Check sheet for the modelled part. Datum: model origin and axes. Units: mm. A direction names the side the tool comes from. Give positions to 0.01 mm unless a question says otherwise; leave off trailing zeros. Loops run counter-clockwise (first coordinate to the right, second up) from the corner with the lowest first, then second, coordinate; pieces in that order, holes last. Notation, with made-up numbers: M 56.5,17.5 L 73.5,17.5 A25 cw 73.5,38.5 Z; hole C 45,62 d11. An arc over 180 degrees is marked long. Write each question's results on one line, items separated by ' | '. Start each with the question number.
1. Sectioned sample at A-A on z = 0. Record the cut outline in (x, y).
2. Sectioned sample at B-B on x = 0. Record the cut outline in (y, z), and give its area (3 significant figures).
3. Tool access check on faces 4 (the cylindrical face through (0.9, 5.92, 2.86)), 5 (the flat face through (0, 0, 0)). Record the directions out of +Z, -Z, +X, -X, +Y, -Y that give a thin tool (end or side, any length) a straight path to the whole face; none if there is none.
4. Draft check along Z on faces 1 (the cylindrical face through (1.802, 59.328, 5.723)), 2 (the flat face through (0, 130, 0)), 3 (the cylindrical face through (0.14, 117.315, 0.596)). Enter one of: pulls with the +Z half, pulls with the -Z half, needs draft (parallel to the pull), parting line crosses it, or undercut.
5. Sectioned sample at D-D on y = 105. Record the cut outline in (x, z), and give its area (3 significant figures).
6. Material ranges on line 1 along Y through (x, z) = (4.5, 0); line 2 along Y through (x, z) = (-1.5, 0); line 3 along Z through (x, y) = (3, 120), recorded low to high.
7. Sectioned sample at C-C on y = 120. Record the cut outline in (x, z).
8. Go/stop test with flat-tipped pins: pin 1 (1.5 mm diameter, centred on y = 61.5, z = -2, fed in from -X); pin 2 (12 mm diameter, centred on y = 111, z = -7.5, fed in from +X); pin 3 (1 mm diameter, centred on y = 14.5, z = 6, fed in from +X). Record where each tip stops, or that it passes through.
```python
from build123d import *

# Parameters (mm, degrees)
TIP_PIN_SKETCH_6_R        = 3
TIP_PIN_6X12_DEPTH        = 12
SHAFT_SKETCH_12_R         = 6
SHAFT_12X96_DEPTH         = 96
HEAD_SKETCH_20_R          = 10
HEAD_20X22_DEPTH          = 22
CROSS_HOLE_SKETCH_5_5_R   = 2.75
CROSS_HOLE_5_5_DEPTH      = 11
HEAD_CHAMFER_1_15X45_SIZE = 1.15


with BuildPart() as part:
    # Tip Pin Sketch Ø6 → Tip Pin Ø6x12 (new body)
    with BuildSketch(Plane(origin=(0, 0, 0), x_dir=(1, 0, 0), z_dir=(0, 1, 0))):
        with Locations(Location((0, 0, 0), (0, 0, 270))):
            Circle(TIP_PIN_SKETCH_6_R)
    extrude(amount=TIP_PIN_6X12_DEPTH)

    # Shaft Sketch Ø12 → Shaft Ø12x96 (add)
    with BuildSketch(Plane(origin=(0, 12, 0), x_dir=(1, 0, 0), z_dir=(0, 1, 0))):
        with Locations(Location((0, 0, 0), (0, 0, 270))):
            Circle(SHAFT_SKETCH_12_R)
    extrude(amount=SHAFT_12X96_DEPTH)

    # Head Sketch Ø20 → Head Ø20x22 (add)
    with BuildSketch(Plane(origin=(0, 108, 0), x_dir=(1, 0, 0), z_dir=(0, 1, 0))):
        with Locations(Location((0, 0, 0), (0, 0, 270))):
            Circle(HEAD_SKETCH_20_R)
    extrude(amount=HEAD_20X22_DEPTH)

    # Cross Hole Sketch Ø5.5 → Cross Hole Ø5.5 (cut, symmetric)
    with BuildSketch(Plane(origin=(0, 0, 0), x_dir=(0, 0, -1), z_dir=(1, 0, 0))):
        with Locations((0, 120)):
            Circle(CROSS_HOLE_SKETCH_5_5_R)
    extrude(amount=CROSS_HOLE_5_5_DEPTH, both=True, mode=Mode.SUBTRACT)

    # Head Chamfer 1.15x45°
    head_chamfer_1_15x45_edges = [part.edges().sort_by_distance(p)[0] for p in [
        (0, 130, -10),
    ]]
    chamfer(head_chamfer_1_15x45_edges, length=HEAD_CHAMFER_1_15X45_SIZE)


solid = part.part
```
Output values:
1) outline: M -10,108 L -6,108 L -6,12 L -3,12 L -3,0 L 3,0 L 3,12 L 6,12 L 6,108 L 10,108 L 10,117.25 L -10,117.25 Z; M -10,122.75 L 10,122.75 L 10,128.85 L 8.85,130 L -8.85,130 L -10,128.85 Z
2) outline: M 0,-3 L 12,-3 L 12,-6 L 108,-6 L 108,-10 L 128.85,-10 L 130,-8.85 L 130,8.85 L 128.85,10 L 108,10 L 108,6 L 12,6 L 12,3 L 0,3 Z; hole C 120,0 d5.5 | area: 1,640 mm2
3) face 4: -Y | face 5: +Z, -Z, +X, -X, -Y
4) face 1: parting line crosses it | face 2: needs draft | face 3: undercut
5) outline: C 0,0 d12 | area: 113 mm2
6) line 1: 12 to 117.25, 122.75 to 130 | line 2: 0 to 117.25, 122.75 to 130 | line 3: -9.54 to -2.75, 2.75 to 9.54
7) outline: M -9.61,-2.75 A10 ccw 9.61,-2.75 Z; M -9.61,2.75 L 9.61,2.75 A10 ccw Z
8) pin 1: x = -5.87 | pin 2: x = 9.89 | pin 3: x = 2.4
